from build123d import *

# Parameters (mm, degrees)
SKETCH_1_W          = 494.5
SKETCH_1_H          = 1168
SKETCH_1_R          = 3.25
EXTRUDE_1_DEPTH     = 2
SKETCH_3_R          = 1.15
SKETCH_3_R_2        = 11.5
SKETCH_3_R_3        = 11.25
CUT_EXTRUDE_2_DEPTH = 10


with BuildPart() as part:
    # 草图1 → 凸台-拉伸1 (new body)
    with BuildSketch(Plane.XY):
        Rectangle(SKETCH_1_W, SKETCH_1_H)
        with Locations((-237.25, 0)):
            Circle(SKETCH_1_R, mode=Mode.SUBTRACT)
        with Locations((-237.25, -126)):
            Circle(SKETCH_1_R, mode=Mode.SUBTRACT)
        with Locations((-237.25, -252)):
            Circle(SKETCH_1_R, mode=Mode.SUBTRACT)
        with Locations((-237.25, -378)):
            Circle(SKETCH_1_R, mode=Mode.SUBTRACT)
        with Locations((-237.25, -504)):
            Circle(SKETCH_1_R, mode=Mode.SUBTRACT)
        with Locations((0, -574)):
            Circle(SKETCH_1_R, mode=Mode.SUBTRACT)
        with Locations(Location((0, 574, 0), (0, 0, 180))):
            Circle(SKETCH_1_R, mode=Mode.SUBTRACT)
        with Locations(Location((-237.25, 504, 0), (0, 0, 180))):
            Circle(SKETCH_1_R, mode=Mode.SUBTRACT)
        with Locations(Location((-237.25, 378, 0), (0, 0, 180))):
            Circle(SKETCH_1_R, mode=Mode.SUBTRACT)
        with Locations(Location((-237.25, 252, 0), (0, 0, 180))):
            Circle(SKETCH_1_R, mode=Mode.SUBTRACT)
        with Locations(Location((-237.25, 126, 0), (0, 0, 180))):
            Circle(SKETCH_1_R, mode=Mode.SUBTRACT)
        with Locations((237.25, 126)):
            Circle(SKETCH_1_R, mode=Mode.SUBTRACT)
        with Locations((237.25, 252)):
            Circle(SKETCH_1_R, mode=Mode.SUBTRACT)
        with Locations((237.25, 378)):
            Circle(SKETCH_1_R, mode=Mode.SUBTRACT)
        with Locations((237.25, 504)):
            Circle(SKETCH_1_R, mode=Mode.SUBTRACT)
        with Locations(Location((237.25, -504, 0), (0, 0, 180))):
            Circle(SKETCH_1_R, mode=Mode.SUBTRACT)
        with Locations(Location((237.25, -378, 0), (0, 0, 180))):
            Circle(SKETCH_1_R, mode=Mode.SUBTRACT)
        with Locations(Location((237.25, -252, 0), (0, 0, 180))):
            Circle(SKETCH_1_R, mode=Mode.SUBTRACT)
        with Locations(Location((237.25, -126, 0), (0, 0, 180))):
            Circle(SKETCH_1_R, mode=Mode.SUBTRACT)
        with Locations(Location((237.25, 0, 0), (0, 0, 180))):
            Circle(SKETCH_1_R, mode=Mode.SUBTRACT)
        with Locations((-210, 574)):
            Circle(SKETCH_1_R, mode=Mode.SUBTRACT)
        with Locations((210, 574)):
            Circle(SKETCH_1_R, mode=Mode.SUBTRACT)
        with Locations(Location((210, -574, 0), (0, 0, 180))):
            Circle(SKETCH_1_R, mode=Mode.SUBTRACT)
        with Locations(Location((-210, -574, 0), (0, 0, 180))):
            Circle(SKETCH_1_R, mode=Mode.SUBTRACT)
    extrude(amount=EXTRUDE_1_DEPTH)

    # 草图3 → 切除-拉伸2 (cut)
    with BuildSketch(Plane(origin=(0, 0, 0), x_dir=(-1, 0, 0), z_dir=(0, 0, -1))):
        with Locations((-48.25, 145.832522251)):
            Circle(SKETCH_3_R)
        with Locations((-10.25, 185.832522251)):
            Circle(SKETCH_3_R_2)
        with Locations((-32.25, 145.832522251)):
            Circle(SKETCH_3_R)
        with Locations((11.75, 145.832522251)):
            Circle(SKETCH_3_R)
        with Locations((27.75, 145.832522251)):
            Circle(SKETCH_3_R)
        with Locations((71.75, 145.832522251)):
            Circle(SKETCH_3_R)
        with Locations((49.75, 270.832522251)):
            Circle(SKETCH_3_R_2)
        with Locations((27.75, 230.832522251)):
            Circle(SKETCH_3_R)
        with Locations((71.75, 230.832522251)):
            Circle(SKETCH_3_R)
        with Locations((-130.25, 185.832522251)):
            Circle(SKETCH_3_R_2)
        with Locations((-152.25, 145.832522251)):
            Circle(SKETCH_3_R)
        with Locations((-108.25, 145.832522251)):
            Circle(SKETCH_3_R)
        with Locations((-70.25, 185.832522251)):
            Circle(SKETCH_3_R_2)
        with Locations((-92.25, 145.832522251)):
            Circle(SKETCH_3_R)
        with Locations((-152.25, 230.832522251)):
            Circle(SKETCH_3_R)
        with Locations((-108.25, 230.832522251)):
            Circle(SKETCH_3_R)
        with Locations((-70.25, 270.832522251)):
            Circle(SKETCH_3_R_2)
        with Locations((-92.25, 230.832522251)):
            Circle(SKETCH_3_R)
        with Locations((-48.25, 230.832522251)):
            Circle(SKETCH_3_R)
        with Locations((-10.25, 270.832522251)):
            Circle(SKETCH_3_R_2)
        with Locations((-32.25, 230.832522251)):
            Circle(SKETCH_3_R)
        with Locations((11.75, 230.832522251)):
            Circle(SKETCH_3_R)
        with Locations((-40.25, 95.832522251)):
            Circle(SKETCH_3_R_2)
        with Locations((-62.25, 47.832522251)):
            Circle(SKETCH_3_R)
        with Locations((-18.25, 47.832522251)):
            Circle(SKETCH_3_R)
        with Locations((-130.25, 270.832522251)):
            Circle(SKETCH_3_R_2)
        with Locations((49.75, 185.832522251)):
            Circle(SKETCH_3_R_3)
    extrude(amount=-CUT_EXTRUDE_2_DEPTH, mode=Mode.SUBTRACT)


solid = part.part
Check sheet for the modelled part. Datum: model origin and axes. Units: mm. Round coordinates to 2 decimals unless told otherwise and drop trailing zeros. Answer as CSV lines item,"result". Start each with the question number.
Item 1: Scan lines: line 1 (Y direction, x = 108.25, z = 1.2); line 2 (X direction, y = -252, z = 1.2); line 3 (Y direction, x = 130.25, z = 0.65). Record each from-to range of solid material in increasing order. Write a range as [from, to].
Item 2: Depth check by flat-ended pin: P1, Ø4, axis at x = 210, y = -574, coming from the +Z side (3 decimals). Enter the tip coordinate at first touch or a pass-through.
Item 3: Release check for a two-part mould opening along Y. For faces 1 (the cylindrical face through (42.743, 84.606, 0.986)), 2 (the flat face through (-3, 8, 0)) record: +Y half, -Y half, draft (parallel to the pull), parting line (faces both ways), or undercut.
Report:
1,line 1,"y = [-584, 144.68], [146.98, 229.68], [231.98, 584]"
1,line 2,"x = [-247.25, -240.5], [-234, 234], [240.5, 247.25]"
1,line 3,"y = [-584, 174.33], [197.33, 259.33], [282.33, 584]"
2,P1,"passes through"
3,face 1,"undercut"
3,face 2,"draft"
